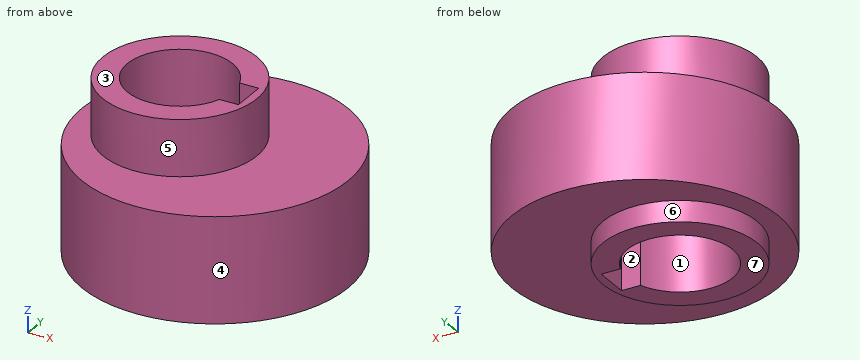
```python
from build123d import *

# Parameters (mm, degrees)
SKETCH1_R           = 11
BOSS_EXTRUDE1_DEPTH = 26
BOSS_EXTRUDE2_START = -8
SKETCH2_R           = 19
BOSS_EXTRUDE2_DEPTH = 15
CUT_EXTRUDE1_DEPTH  = 43


with BuildPart() as part:
    # Sketch1 → Boss-Extrude1 (new body)
    with BuildSketch(Plane.XY):
        with Locations(Location((0, 0, 0), (0, 0, 180))):
            Circle(SKETCH1_R)
    extrude(amount=BOSS_EXTRUDE1_DEPTH)

    # Sketch2 → Boss-Extrude2 (add)
    with BuildSketch(Plane.XY.offset(26).offset(BOSS_EXTRUDE2_START)):
        with Locations((5, 0)):
            Circle(SKETCH2_R)
    extrude(amount=-BOSS_EXTRUDE2_DEPTH)

    # Sketch3 → Cut-Extrude1 (cut)
    with BuildSketch(Plane.XY.offset(26)):
        with BuildLine():
            Line((7.071067812, 2.5), (9.8, 2.5))
            Line((9.8, 2.5), (9.8, -2.5))
            Line((9.8, -2.5), (7.071067812, -2.5))
            ThreePointArc((7.071067812, -2.5), (-7.5, 0), (7.071067812, 2.5))
        make_face()
    extrude(amount=-CUT_EXTRUDE1_DEPTH, mode=Mode.SUBTRACT)


solid = part.part
```
Read the model definition and answer for the solid it produces. Units are mm, in the model's axes. Face numbers are marked on the shaded views. A direction names the side the tool comes from. Give positions to 0.01 mm unless a question says otherwise; leave off trailing zeros. Order: outer loops, then holes, each group sorted by start corner. A loop starts at its lowest first (then second) coordinate and runs counter-clockwise, first axis right, second up. Notation, with made-up numbers: (-33.75, -33.5) -> (0.25, -33.5) arc R29 cw to (0.25, -13.5) -> close; hole circle Ø2 at (12.5, 52). An arc over 180 degrees is marked (long way). One line per item, written item: value. Start each with the question number.
(1) The part is cut by section B-B (z = 24.25). Determine the outline of the cut face in (x, y), and give its area (3 significant figures).
(2) Flat-ended cylindrical pins translate along their axes: P1, Ø2, axis at y = 2, z = 9.5, coming from the +X side; P2, Ø8, axis at x = 7, z = 19.5, coming from the +Y side; P3, Ø1, axis at x = 16, z = 15.5, coming from the +Y side; P4, Ø8, axis at x = -9, y = 2, coming from the -Z side. Find the tip coordinate at first contact, or state that the pin passes through.
(3) The part is cut by section D-D (y = 8.5). Determine the outline of the cut face in (x, z).
(4) For a pull along Y with two mould halves and no side action, classify the marked faces 1, 2, 3 and 4 as released by +Y, released by -Y, zero draft, split by the parting line, or undercut.
(5) The part is cut by section A-A (y = 0). Determine the outline of the cut face in (x, z), and give its area (3 significant figures).
(6) A tool of negligible diameter and unlimited length cuts with its end or side. For the marked faces 5, 6 and 7, from which of +Z, -Z, +X, -X, +Y, -Y can it reach the whole face along a straight path? Write none if from no direction.
(7) Straight lines are drawn through the part: L1, parallel to Y at x = 0, z = 19.5; L2, parallel to Z at x = 21, y = -5; L3, parallel to Y at x = -0.5, z = 8. For each, find the intervals that lie inside material, in ascending order.
(8) The part is cut by section C-C (x = 6.5). Determine the outline of the cut face in (y, z), and give its area (3 significant figures).
Taken from the geometry:
1. outline: circle Ø22 at (0, 0); hole (7.07, -2.5) -> (9.8, -2.5) -> (9.8, 2.5) -> (7.07, 2.5) arc R7.5 ccw (long way) to start
1. area: 191 mm^2
2. P1: x = 23.97
2. P2: y = 19
2. P3: y = 15.84
2. P4: z = 0
3. outline: (-11.99, 3) -> (-6.98, 3) -> (-6.98, 0) -> (6.98, 0) -> (6.98, 3) -> (21.99, 3) -> (21.99, 18) -> (6.98, 18) -> (6.98, 26) -> (-6.98, 26) -> (-6.98, 18) -> (-11.99, 18) -> close
4. face 1: undercut
4. face 2: undercut
4. face 3: zero draft
4. face 4: split by the parting line
5. outline: (-14, 3) -> (-11, 3) -> (-11, 0) -> (-7.5, 0) -> (-7.5, 26) -> (-11, 26) -> (-11, 18) -> (-14, 18) -> close; (9.8, 0) -> (11, 0) -> (11, 3) -> (24, 3) -> (24, 18) -> (11, 18) -> (11, 26) -> (9.8, 26) -> close
5. area: 362 mm^2
6. face 5: +Z
6. face 6: -Z
6. face 7: -Z, +X, -X, +Y, -Y
7. L1: -11 to -7.5, 7.5 to 11
7. L2: 3 to 18
7. L3: -18.19 to -7.48, 7.48 to 18.19
8. outline: (-18.94, 3) -> (-8.87, 3) -> (-8.87, 0) -> (-3.74, 0) -> (-3.74, 26) -> (-8.87, 26) -> (-8.87, 18) -> (-18.94, 18) -> close; (3.74, 0) -> (8.87, 0) -> (8.87, 3) -> (18.94, 3) -> (18.94, 18) -> (8.87, 18) -> (8.87, 26) -> (3.74, 26) -> close
8. area: 569 mm^2
